```python
from build123d import *

# Parameters (mm, degrees)
EXTRUDE_1_DEPTH          = 25
CHAMFER_1_SIZE           = 10
CUT_EXTRUDE_1_DEPTH      = 1655.063178963
CUT_EXTRUDE_1_DEPTH_BACK = 1655.063178963
SKETCH_2_R               = 20


with BuildPart() as part:
    # 草图1 → 凸台-拉伸1 (new body)
    with BuildSketch(Plane.XY):
        Polygon((160, -280), (0, -280), (0, 0), (1630, 0), (1630, -280), (1240, -280), (1240, -115), (160, -115), align=None)
    extrude(amount=EXTRUDE_1_DEPTH)

    # 倒角1
    chamfer_1_edges = [part.edges().sort_by_distance(p)[0] for p in [
        (0, -280, 12.5),
        (0, 0, 12.5),
        (1630, 0, 12.5),
        (1630, -280, 12.5),
    ]]
    chamfer(chamfer_1_edges, length=CHAMFER_1_SIZE)

    # 草图2 → 切除-拉伸1 (cut, two sides: drawn at the far end of the back side and taken through both)
    with BuildSketch(Plane.XY.offset(25).offset(-CUT_EXTRUDE_1_DEPTH_BACK)):
        with Locations((50, -80)):
            Circle(SKETCH_2_R)
        with Locations((1580, -80)):
            Circle(SKETCH_2_R)
    extrude(amount=CUT_EXTRUDE_1_DEPTH + CUT_EXTRUDE_1_DEPTH_BACK, mode=Mode.SUBTRACT)


solid = part.part
```
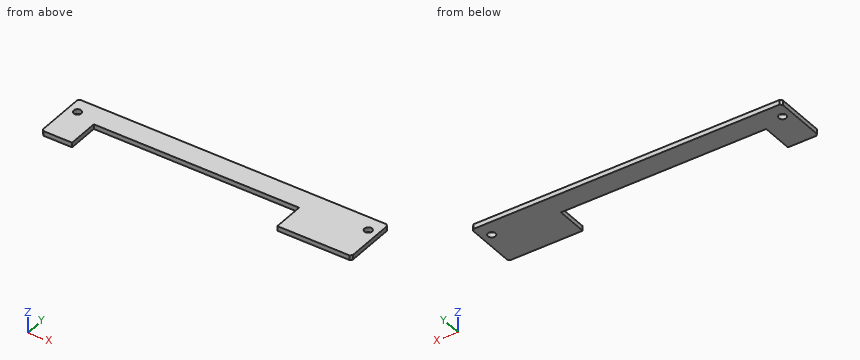
Geometry check sheet. Reference: the model listing, model coordinates, mm. Give positions to 0.01 mm unless a question says otherwise; leave off trailing zeros. Order: outer loops, then holes, each group sorted by start corner. A loop starts at its lowest first (then second) coordinate and runs counter-clockwise, first axis right, second up. Notation, with made-up numbers: (53, 81.5) - (103, 81.5) arc R19 ccw to (103, 88.5) - close; hole circle Ø5 at (30.5, 76). An arc over 180 degrees is marked (long way). Answer in a Markdown table with one row per item. Add a question column.
Q1. Gauge pin test, flat end, axial feed: pin 1 (1 mm diameter, centred on x = 922, z = 17.5, fed in from -Y). Record the tip position at first contact, or that the pin passes through.
Q2. Cross-section at B-B, the plane x = 50. Enter the section's corners in (y, z), then the cut area to 3 significant figures.
Q3. Material ranges on probe 1 along X at (y, z) = (-80, 19.5); probe 2 along X at (y, z) = (-202.5, 22.25); probe 3 along Y at (x, z) = (1580, 19.5), recorded low to high. Write a range as from..to.
Q4. Cross-section at D-D, the plane y = -232. Enter the section's corners in (x, z), then the cut area to 4 significant figures.
Q5. Cross-section at C-C, the plane z = 18. Enter the section's corners in (x, y).
Q6. Cross-section at A-A, the plane y = -80. Enter the section's corners in (x, z), then the cut area to 4 significant figures.
Check values:
| question | item | result |
|---|---|---|
| 1 | pin 1 | stops at y = -115 |
| 2 | outline | (-280, 0) - (-100, 0) - (-100, 25) - (-280, 25) - close; (-60, 0) - (0, 0) - (0, 25) - (-60, 25) - close |
| 2 | area | 6,000 mm^2 |
| 3 | probe 1 | x = 0..30, 70..1560, 1600..1630 |
| 3 | probe 2 | x = 0..160, 1240..1630 |
| 3 | probe 3 | y = -280..-100, -60..0 |
| 4 | outline | (0, 0) - (160, 0) - (160, 25) - (0, 25) - close; (1240, 0) - (1630, 0) - (1630, 25) - (1240, 25) - close |
| 4 | area | 13,750 mm^2 |
| 5 | outline | (0, -270) - (10, -280) - (160, -280) - (160, -115) - (1240, -115) - (1240, -280) - (1620, -280) - (1630, -270) - (1630, -10) - (1620, 0) - (10, 0) - (0, -10) - close; hole circle Ø40 at (50, -80); hole circle Ø40 at (1580, -80) |
| 6 | outline | (0, 0) - (30, 0) - (30, 25) - (0, 25) - close; (70, 0) - (1560, 0) - (1560, 25) - (70, 25) - close; (1600, 0) - (1630, 0) - (1630, 25) - (1600, 25) - close |
| 6 | area | 38,750 mm^2 |
